from build123d import *

# Parameters (mm, degrees)
SKETCH1_R             = 10
BOSS_EXTRUDE1_DEPTH   = 700
M8_TAPPED_HOLE1_D     = 6.8
M8_TAPPED_HOLE1_DEPTH = 19.75
M8_TAPPED_HOLE1_TIP   = 2.042926105
M8_TAPPED_HOLE2_D     = 6.8
M8_TAPPED_HOLE2_DEPTH = 19.75
M8_TAPPED_HOLE2_TIP   = 2.042926105


with BuildPart() as part:
    # Sketch1 → Boss-Extrude1 (new body)
    with BuildSketch(Plane(origin=(0, 0, 0), x_dir=(1, 0, 0), z_dir=(0, 1, 0))):
        with Locations(Location((0, 0, 0), (0, 0, 270))):
            Circle(SKETCH1_R)
    extrude(amount=BOSS_EXTRUDE1_DEPTH)

    # M8 Tapped Hole1
    with Locations(Plane(origin=(0, 700, 0), x_dir=(1, 0, 0), z_dir=(0, 1, 0))):
        with Locations((0, 0)):
            Hole(M8_TAPPED_HOLE1_D / 2, depth=M8_TAPPED_HOLE1_DEPTH)
            with Locations((0, 0, -(M8_TAPPED_HOLE1_DEPTH + M8_TAPPED_HOLE1_TIP / 2))):  # 118° drill point
                Cone(0, M8_TAPPED_HOLE1_D / 2, M8_TAPPED_HOLE1_TIP, mode=Mode.SUBTRACT)

    # M8 Tapped Hole2
    with Locations(Plane(origin=(0, 0, 0), x_dir=(-1, 0, 0), z_dir=(0, -1, 0))):
        with Locations((0, 0)):
            Hole(M8_TAPPED_HOLE2_D / 2, depth=M8_TAPPED_HOLE2_DEPTH)
            with Locations((0, 0, -(M8_TAPPED_HOLE2_DEPTH + M8_TAPPED_HOLE2_TIP / 2))):  # 118° drill point
                Cone(0, M8_TAPPED_HOLE2_D / 2, M8_TAPPED_HOLE2_TIP, mode=Mode.SUBTRACT)


solid = part.part
For this review, take the finished solid that the model builds, in its own axes (mm). Coordinates: 2 decimals unless noted, no trailing zeros. Order: outer loops, then holes, each group sorted by start corner. A loop starts at its lowest first (then second) coordinate and runs counter-clockwise, first axis right, second up. Notation, with made-up numbers: (-15, 6.25) - (21, 6.25) arc R30 cw to (21, 35.25) - close; hole circle Ø2 at (6, 82). An arc over 180 degrees is marked (long way). Use one line per item in the form item = value.
Q1. Consider section B-B (x = 6.75). Give the boundary of the cut face in (y, z), then the cut area to 3 significant figures.
Checked values:
outline = (0, -7.38) - (700, -7.38) - (700, 7.38) - (0, 7.38) - close
area = 10,300 mm2
Q2. For probe 1 along X at (y, z) = (508.5, 0); probe 2 along Z at (x, y) = (-2.5, 36); probe 3 along X at (y, z) = (465, 1.75), list the stretches that pass through material, from the lowest coordinate up. Write a range as from..to.
Checked values:
probe_1 = -10..10
probe_2 = -9.68..9.68
probe_3 = -9.85..9.85
Q3. Consider section A-A (y = 64). Give the boundary of the cut face in (x, z).
Checked values:
outline = circle Ø20 at (0, 0)
Q4. For P1, Ø8, axis at y = 344, z = -5.5, coming from the +X side; P2, Ø4, axis at x = -3.5, y = 231, coming from the -Z side; P3, Ø4, axis at x = 0, z = 0, coming from the +Y side, all flat-tipped, find the tip position at first contact; note any pin that passes through.
Checked values:
P1 = 9.89
P2 = -9.89
P3 = 679.41
